Verification items for the finished model (mm, model axes). A direction names the side the tool comes from. Round coordinates to 2 decimals unless told otherwise and drop trailing zeros. Order: outer loops, then holes, each group sorted by start corner. A loop starts at its lowest first (then second) coordinate and runs counter-clockwise, first axis right, second up. Notation, with made-up numbers: (16, 34) -> (41, 34) arc R24 ccw to (41, 52) -> close; hole circle Ø5 at (46, 8). An arc over 180 degrees is marked (long way). Return JSON: item names as keys, results as strings. Group by question number.
1) Section check C-C on x = 280.5. Enter the section's corners in (y, z).
2) Section check B-B on z = 3.3. Enter the section's corners in (x, y), plus the area to 3 significant figures.
3) Section check A-A on y = 165. Enter the section's corners in (x, z), plus the area to 3 significant figures.
4) Scan lines: L1, parallel to Y at x = 186.5, z = 1.3; L2, parallel to Y at x = 270, z = 1.5; L3, parallel to X at y = 137.5, z = 4.6. Record each from-to range of solid material in increasing order.
5) Depth check by flat-ended pin: pin 1 (12 mm diameter, centred on x = 99, y = 81, fed in from -Z). Enter the tip coordinate at first touch or a pass-through.
6) Tool access check on faces 3 (the cylindrical face through (87.522, 167.034, 2.465)), 4 (the flat face through (193, 277, 0)). Record the directions out of +Z, -Z, +X, -X, +Y, -Y that give a thin tool (end or side, any length) a straight path to the whole face; none if there is none.
7) Draft check along Y on faces 1 (the flat face through (193, 277, 5)), 2 (the cylindrical face through (292.478, 162.966, 2.465)). Enter one of: pulls with the +Y half, pulls with the -Y half, needs draft (parallel to the pull), parting line crosses it, or undercut.
```python
from build123d import *

# Parameters (mm, degrees)
SKETCH_1_W          = 380
SKETCH_1_H          = 330
EXTRUDE_1_DEPTH     = 5
CUT_EXTRUDE_1_DEPTH = 10
EXTRUDE_2_DEPTH     = 5


with BuildPart() as part:
    # 草图1 → 凸台-拉伸1 (new body)
    with BuildSketch(Plane.XY):
        with Locations((190, 165)):
            Rectangle(SKETCH_1_W, SKETCH_1_H)
    extrude(amount=EXTRUDE_1_DEPTH)

    # 草图2 → 切除-拉伸1 (cut)
    with BuildSketch(Plane(origin=(0, 0, 0), x_dir=(-1, 0, 0), z_dir=(0, 0, -1))):
        with BuildLine():
            Line((-210, 72.5), (-170, 72.5))
            ThreePointArc((-170, 72.5), (-77.5, 165), (-170, 257.5))
            Line((-170, 257.5), (-210, 257.5))
            ThreePointArc((-210, 257.5), (-302.5, 165), (-210, 72.5))
        make_face()
    extrude(amount=-CUT_EXTRUDE_1_DEPTH, mode=Mode.SUBTRACT)

    # 草图3 → 凸台-拉伸2 (add)
    with BuildSketch(Plane(origin=(0, 0, 0), x_dir=(-1, 0, 0), z_dir=(0, 0, -1))):
        with BuildLine():
            ThreePointArc((-210, 257.5), (-302.5, 165), (-210, 72.5))
            Line((-210, 72.5), (-200, 72.5))
            ThreePointArc((-200, 72.5), (-292.5, 165), (-200, 257.5))
            Line((-200, 257.5), (-210, 257.5))
        make_face()
        with BuildLine():
            ThreePointArc((-180, 257.5), (-87.5, 165), (-180, 72.5))
            Line((-180, 72.5), (-170, 72.5))
            ThreePointArc((-170, 72.5), (-77.5, 165), (-170, 257.5))
            Line((-170, 257.5), (-180, 257.5))
        make_face()
    extrude(amount=-EXTRUDE_2_DEPTH)


solid = part.part
```
Check result:
{
 "1": {"outline": "(0, 0) -> (119.44, 0) -> (119.44, 5) -> (0, 5) -> close; (210.56, 0) -> (330, 0) -> (330, 5) -> (210.56, 5) -> close"},
 "2": {"outline": "(0, 0) -> (380, 0) -> (380, 330) -> (0, 330) -> close; hole (180, 72.5) -> (200, 72.5) arc R92.5 ccw to (200, 257.5) -> (180, 257.5) arc R92.5 ccw to start", "area": "94,800 mm^2"},
 "3": {"outline": "(0, 0) -> (87.5, 0) -> (87.5, 5) -> (0, 5) -> close; (292.5, 0) -> (380, 0) -> (380, 5) -> (292.5, 5) -> close", "area": "875 mm^2"},
 "4": {"L1": "0 to 72.5, 257.5 to 330", "L2": "0 to 104.53, 225.47 to 330", "L3": "0 to 91.68, 288.32 to 380"},
 "5": {"pin 1": "z = 0"},
 "6": {"face 3": "+Z, -Z", "face 4": "-Z, +X, -X, +Y, -Y"},
 "7": {"face 1": "needs draft", "face 2": "undercut"}
}
